Answer from the drawing. Dimensions are ordinates in mm from the lowest x, y and z of the part. Round coordinates to 2 decimals unless told otherwise and drop trailing zeros. Order: outer loops, then holes, each group sorted by start corner. A loop starts at its lowest first (then second) coordinate and runs counter-clockwise, first axis right, second up. Notation, with made-up numbers: M 47.25,-15 L 62.25,-15 A30 ccw 62.25,11 Z; hole C -25.5,-4 d7. An arc over 180 degrees is marked long. Write item = value, one per line. Start each with the question number.
(1) A cutting plane is placed at B-B, the plane x = 38. Determine the outline of the cut face in (y, z), and give its area (3 significant figures).
(2) A cutting plane is placed at C-C, the plane z = 6.5. Determine the outline of the cut face in (x, y).
(3) A cutting plane is placed at D-D, the plane x = 15. Determine the outline of the cut face in (y, z).
(4) Straight lines are drawn through the part: probe 1 along Y at (x, z) = (55, 6.5); probe 2 along Y at (x, z) = (15, 3.25); probe 3 along Y at (x, z) = (35, 6.25). For each, find the intervals that lie inside material, in ascending order. Write a range as from..to.
(5) For a pull along X with two mould halves and no side action, classify the marked faces 1, 2, 3 and 4 as released by +X, released by -X, zero draft, split by the parting line, or undercut.
(6) A cutting plane is placed at A-A, the plane y = 15. Determine the outline of the cut face in (x, z), and give its area (3 significant figures).
(7) This flat-tipped pin is pushed along its axis until it touches: pin 1 (6.5 mm diameter, centred on x = 55, y = 15, fed in from +Z). Where does it stop, or does it pass through?
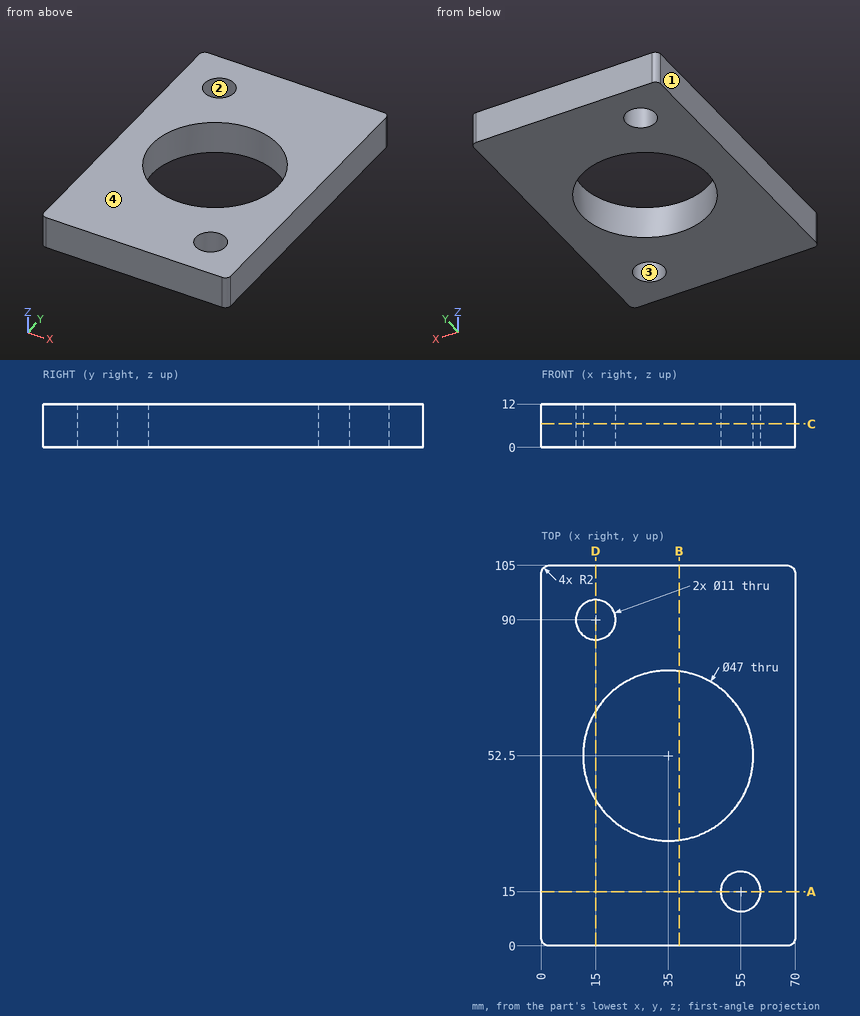
Reported:
q1.outline = M 0,0 L 29.19,0 L 29.19,12 L 0,12 Z; M 75.81,0 L 105,0 L 105,12 L 75.81,12 Z
q1.area = 701 mm²
q2.outline = M 0,2 A2 ccw 2,0 L 68,0 A2 ccw 70,2 L 70,103 A2 ccw 68,105 L 2,105 A2 ccw 0,103 Z; hole C 15,90 d11; hole C 35,52.5 d47; hole C 55,15 d11
q3.outline = M 0,0 L 40.16,0 L 40.16,12 L 0,12 Z; M 64.84,0 L 84.5,0 L 84.5,12 L 64.84,12 Z; M 95.5,0 L 105,0 L 105,12 L 95.5,12 Z
q4.probe_1 = 0..9.5, 20.5..40.16, 64.84..105
q4.probe_2 = 0..40.16, 64.84..84.5, 95.5..105
q4.probe_3 = 0..29, 76..105
q5.face_1 = released by -X
q5.face_2 = undercut
q5.face_3 = undercut
q5.face_4 = zero draft
q6.outline = M 0,0 L 49.5,0 L 49.5,12 L 0,12 Z; M 60.5,0 L 70,0 L 70,12 L 60.5,12 Z
q6.area = 708 mm²
q7.pin_1 = through
